from build123d import *

# Parameters (mm, degrees)
EXTRUDE_1_DEPTH = 10


with BuildPart() as part:
    # 草图2 → 拉伸-薄壁1 (new, symmetric)
    with BuildSketch(Plane.XY):
        with BuildLine():
            Line((-101.625, -635), (-101.625, 0))
            ThreePointArc((-101.625, 0), (0, 101.625), (101.625, 0))
            Line((101.625, 0), (101.625, -635))
            ThreePointArc((101.625, -635), (0, -736.625), (-101.625, -635))
        make_face()
        with BuildLine():
            Line((-91.625, -635), (-91.625, 0))
            ThreePointArc((-91.625, 0), (0, 91.625), (91.625, 0))
            Line((91.625, 0), (91.625, -635))
            ThreePointArc((91.625, -635), (0, -726.625), (-91.625, -635))
        make_face(mode=Mode.SUBTRACT)
    extrude(amount=EXTRUDE_1_DEPTH, both=True)


solid = part.part
Model file for the job. Use its own axes, mm. A direction names the side the tool comes from. Round coordinates to 2 decimals unless told otherwise and drop trailing zeros. Loops run counter-clockwise (first coordinate to the right, second up) from the corner with the lowest first, then second, coordinate; pieces in that order, holes last. Notation, with made-up numbers: (4, 19) -> (33, 19) arc R20 ccw to (33, 51) -> close; hole circle Ø4 at (46, 0.5). An arc over 180 degrees is marked (long way). Answer as CSV lines item,"result". Start each with the question number.
1) Tool access for faces 5 (the face through (2.015, -726.603, 0.14)), 6 (the face through (-101.625, -322, 0)): list every direction of +Z, -Z, +X, -X, +Y, -Y with a clear straight run to the whole face (end or side of a thin tool).
2) Probe line 1 along X through (y, z) = (-496, 5.25) (3 decimals); line 2 along Y through (x, z) = (5, -1.25); line 3 along Y through (x, z) = (71, -3.75). List the from-to ranges inside material, lowest first.
3) Slice it at B-B (x = 0). List the corners of the cut face in (y, z) (3 decimals).
4) Slice it at C-C (z = -3.75). List the corners of the cut face in (x, y) (3 decimals), plus the area to 3 significant figures.
5) Pin check, flat tips, straight feed: P1, Ø6, axis at x = 16, z = -5, coming from the +Y side; P2, Ø1.5, axis at x = -38, z = 6.5, coming from the -Y side; P3, Ø12, axis at x = -18.5, z = 4, coming from the -Y side. Stop position of each tip, or through.
6) Slice it at A-A (y = -530.5). List the corners of the cut face in (x, z) (3 decimals), plus the area to 3 significant figures.
7) Mould opens along X. For faces 1 (the face through (-2.2, 101.6, 0.1)), 2 (the face through (-97, -316, -10)), 3 (the face through (-2.015, 91.603, 0.14)), 4 (the face through (91.625, -313, 0)) say: +X half, -X half, draft (parallel to the pull), parting line (faces both ways), or undercut.
Filled in:
1,face 5,"+Z, -Z"
1,face 6,"+Z, -Z, -X, +Y, -Y"
2,line 1,"x = -101.625 to -91.625, 91.625 to 101.625"
2,line 2,"y = -736.5 to -726.49, 91.49 to 101.5"
2,line 3,"y = -707.71 to -692.91, 57.91 to 72.71"
3,outline,"(-736.625, -10) -> (-726.625, -10) -> (-726.625, 10) -> (-736.625, 10) -> close; (91.625, -10) -> (101.625, -10) -> (101.625, 10) -> (91.625, 10) -> close"
4,outline,"(-101.625, -635) arc R101.625 ccw to (101.625, -635) -> (101.625, 0) arc R101.625 ccw to (-101.625, 0) -> close; hole (-91.625, -635) arc R91.625 ccw to (91.625, -635) -> (91.625, 0) arc R91.625 ccw to (-91.625, 0) -> close"
4,area,"18,800 mm2"
5,P1,"stops at y = 100.79"
5,P2,"stops at y = -729.55"
5,P3,"stops at y = -735.85"
6,outline,"(-101.625, -10) -> (-91.625, -10) -> (-91.625, 10) -> (-101.625, 10) -> close; (91.625, -10) -> (101.625, -10) -> (101.625, 10) -> (91.625, 10) -> close"
6,area,"400 mm2"
7,face 1,"parting line"
7,face 2,"draft"
7,face 3,"undercut"
7,face 4,"undercut"
